For this review, take the finished solid that the model builds, in its own axes (mm). Face numbers are marked on the shaded views. Give positions to 0.01 mm unless a question says otherwise; leave off trailing zeros. Write each loop counter-clockwise with the first axis right and the second up, starting at its lowest first coordinate (ties: lowest second). Pieces come first, ordered by that corner, then holes.
Q1. Mouldability with a two-part tool opening along Z and no side actions: class the marked faces 1, 2 and 3 as released by +Z, released by -Z, zero draft, split by the parting line, or undercut.
Q2. We need section A-A (z = 6). Write out the cut boundary in (x, y), then the cut area to 3 significant figures.
Q3. Insertion check: P1, Ø1, axis at y = 2, z = 2, coming from the -X side; P2, Ø1.5, axis at x = 7.5, z = 5, coming from the +Y side; P3, Ø3, axis at y = -2.5, z = 2, coming from the -X side. Each pin has a flat end and moves straight along its axis. Give the tip position at first contact, or say it passes through.
Q4. For line 1 (Y direction, x = 5, z = 6); line 2 (X direction, y = 0.75, z = 3.5); line 3 (Y direction, x = 6.75, z = 5), list the stretches that pass through material, from the lowest coordinate up.
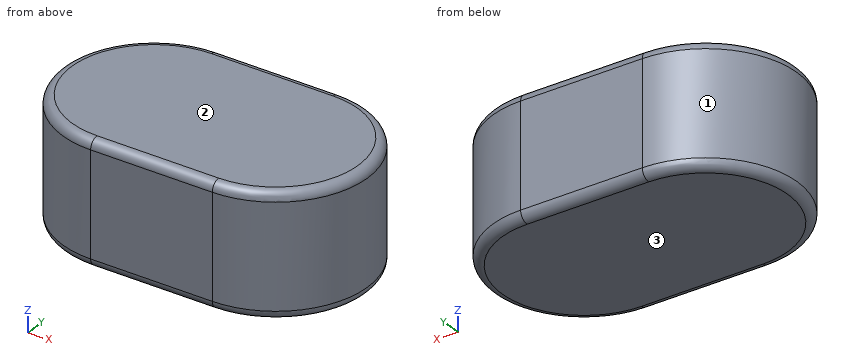
```python
from build123d import *

# Parameters (mm, degrees)
EXTRUDE_523_DEPTH = 8
FILLET_1_R        = 0.6


with BuildPart() as part:
    # 草图1 → Extrude 523 (new body)
    with BuildSketch(Plane.XY):
        with BuildLine():
            Line((-4, 6), (4, 6))
            ThreePointArc((4, 6), (10, 0), (4, -6))
            Line((4, -6), (-4, -6))
            ThreePointArc((-4, -6), (-10, 0), (-4, 6))
        make_face()
    extrude(amount=EXTRUDE_523_DEPTH)

    # 圆角1
    fillet_1_edges = [part.edges().sort_by_distance(p)[0] for p in [
        (10, 0, 8),
        (0, 6, 8),
        (-10, 0, 8),
        (0, 6, 0),
        (10, 0, 0),
        (0, -6, 0),
        (-10, 0, 0),
        (0, -6, 8),
    ]]
    fillet(fillet_1_edges, radius=FILLET_1_R)


solid = part.part
```
Computed:
1. face 1: zero draft
1. face 2: released by +Z
1. face 3: released by -Z
2. outline: (-4, -6) - (4, -6) arc R6 ccw to (4, 6) - (-4, 6) arc R6 ccw to start
2. area: 209 mm2
3. P1: stops at x = -9.81
3. P2: stops at y = 5.33
3. P3: stops at x = -9.92
4. line 1: y = -5.92 to 5.92
4. line 2: x = -9.95 to 9.95
4. line 3: y = -5.33 to 5.33
